CAD build for the part. Positions are in the model's coordinates, mm. Face numbers are marked on the shaded views. A direction names the side the tool comes from. Give positions to 0.01 mm unless a question says otherwise; leave off trailing zeros. Loops run counter-clockwise (first coordinate to the right, second up) from the corner with the lowest first, then second, coordinate; pieces in that order, holes last. Notation, with made-up numbers: M -38,-18 L 7,-18 A11 ccw 7,1 Z; hole C 60,47.25 d6. An arc over 180 degrees is marked long. Answer as CSV lines item,"result".
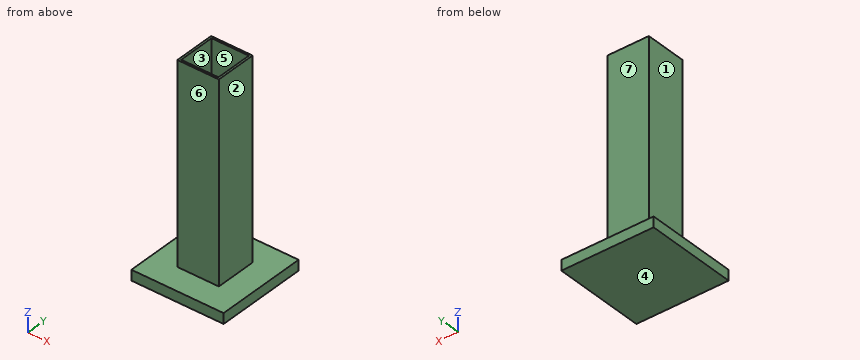
```python
from build123d import *

# Parameters (mm, degrees)
SKETCH1_W           = 445
SKETCH1_H           = 445
BOSS_EXTRUDE1_DEPTH = 50
SKETCH2_W           = 200
SKETCH2_H           = 200
SKETCH2_W_2         = 180
SKETCH2_H_2         = 180
BOSS_EXTRUDE2_DEPTH = 950


with BuildPart() as part:
    # Sketch1 → Boss-Extrude1 (new body)
    with BuildSketch(Plane.XY):
        Rectangle(SKETCH1_W, SKETCH1_H)
    extrude(amount=BOSS_EXTRUDE1_DEPTH)

    # Sketch2 → Boss-Extrude2 (add)
    with BuildSketch(Plane.XY.offset(50)):
        Rectangle(SKETCH2_W, SKETCH2_H)
        Rectangle(SKETCH2_W_2, SKETCH2_H_2, mode=Mode.SUBTRACT)
    extrude(amount=BOSS_EXTRUDE2_DEPTH)


solid = part.part
```
Q1. Cut at B-B (y = 13.5). Write the cut outline in (x, z), and give its area (4 significant figures).
Solution:
outline,"M -222.5,0 L 222.5,0 L 222.5,50 L 100,50 L 100,1000 L 90,1000 L 90,50 L -90,50 L -90,1000 L -100,1000 L -100,50 L -222.5,50 Z"
area,"41,250 mm²"
Q2. Cut at A-A (z = 207). Write the cut outline in (x, y), and give its area (3 significant figures).
Solution:
outline,"M -100,-100 L 100,-100 L 100,100 L -100,100 Z; hole M -90,-90 L 90,-90 L 90,90 L -90,90 Z"
area,"7,600 mm²"
Q3. Cut at D-D (x = -143.5). Write the cut outline in (y, z).
Solution:
outline,"M -222.5,0 L 222.5,0 L 222.5,50 L -222.5,50 Z"
Q4. Which spindle directions (+Z, -Z, +X, -X, +Y, -Y) get a long thin tool onto all of the face, cutting with end or side? Do the marked faces 5, 6 and 7. Say none if no direction does.
Solution:
face 5,"+Z"
face 6,"+Z, +X, -X, -Y"
face 7,"+Z, +X, -X, +Y"
Q5. Wall check: line 1 (X direction, y = 27, z = 319); line 2 (Z direction, x = -29.5, y = 185). Give the ranges that are in metal, low to high. Write a range as [from, to].
Solution:
line 1,"x = [-100, -90], [90, 100]"
line 2,"z = [0, 50]"
Q6. Mould opens along X. For the marked faces 1, 2, 3 and 4 say: released by +X, released by -X, zero draft, split by the parting line, or undercut.
Solution:
face 1,"released by -X"
face 2,"released by +X"
face 3,"undercut"
face 4,"zero draft"
Q7. Pin check, flat tips, straight feed: P1, Ø3, axis at x = -87, y = 55, coming from the -Z side; P2, Ø10, axis at x = 5.5, z = 254.5, coming from the -Y side; P3, Ø1, axis at y = -91.5, z = 126.5, coming from the -X side; P4, Ø4, axis at x = 94.5, z = 713.5, coming from the +Y side. Stop position of each tip, or through.
Solution:
P1,"stops at z = 0"
P2,"stops at y = -100"
P3,"stops at x = -100"
P4,"stops at y = 100"
